Geometry: final body of the model. Coordinates: model frame, mm. Face numbers are marked on the shaded views. A direction names the side the tool comes from. Give positions to 0.01 mm unless a question says otherwise; leave off trailing zeros. Order: outer loops, then holes, each group sorted by start corner. A loop starts at its lowest first (then second) coordinate and runs counter-clockwise, first axis right, second up. Notation, with made-up numbers: (-31, 85) -> (8, 85) arc R33 cw to (8, 119) -> close; hole circle Ø5 at (74.25, 31). An arc over 180 degrees is marked (long way). One line per question, with ' | ' between items.
from build123d import *

# Parameters (mm, degrees)
SKETCH_1_R      = 20
SKETCH_1_R_2    = 14
EXTRUDE_1_DEPTH = 4
SKETCH_2_W      = 40
SKETCH_2_H      = 18
EXTRUDE_2_DEPTH = 2
SKETCH_3_W      = 2
SKETCH_3_H      = 18
EXTRUDE_3_DEPTH = 53
SKETCH_4_W      = 2
SKETCH_4_H      = 18
EXTRUDE_4_DEPTH = 18


with BuildPart() as part:
    # 草图1 → 凸台-拉伸1 (new, symmetric)
    with BuildSketch(Plane.XY):
        Circle(SKETCH_1_R)
        Circle(SKETCH_1_R_2, mode=Mode.SUBTRACT)
    extrude(amount=EXTRUDE_1_DEPTH, both=True)

    # 草图2 → 凸台-拉伸2 (add)
    with BuildSketch(Plane(origin=(0, 0, -4), x_dir=(-1, 0, 0), z_dir=(0, 0, -1))):
        with Locations((37.860571099, 0)):
            Rectangle(SKETCH_2_W, SKETCH_2_H)
    extrude(amount=-EXTRUDE_2_DEPTH)

    # 草图3 → 凸台-拉伸3 (add)
    with BuildSketch(Plane(origin=(0, 0, -4), x_dir=(-1, 0, 0), z_dir=(0, 0, -1))):
        with Locations((56.860571099, 0)):
            Rectangle(SKETCH_3_W, SKETCH_3_H)
    extrude(amount=EXTRUDE_3_DEPTH)

    # 草图4 → 凸台-拉伸4 (add)
    with BuildSketch(Plane.ZY.offset(57.860571099)):
        with Locations((-56, 0)):
            Rectangle(SKETCH_4_W, SKETCH_4_H)
    extrude(amount=EXTRUDE_4_DEPTH)


solid = part.part
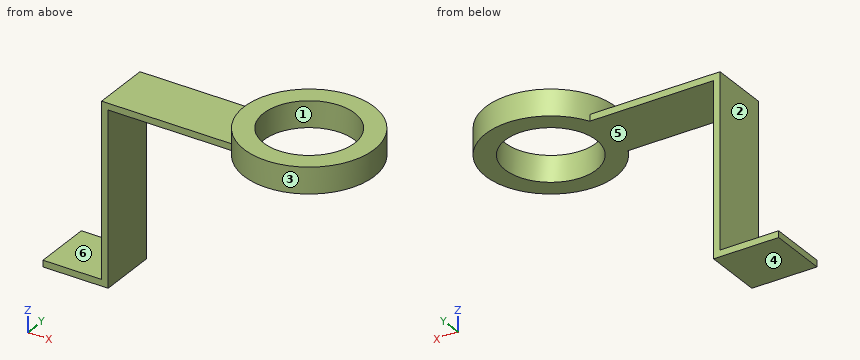
1) Material intervals for probe 1 along Y at (x, z) = (0, -1); probe 2 along Z at (x, y) = (-60, 3); probe 3 along X at (y, z) = (5, -32), sorted ascending. Write a range as from..to.
Check result:
probe 1: y = -20..-14, 14..20 | probe 2: z = -57..-55 | probe 3: x = -57.86..-55.86
2) Section B-B on x = 0. Return loops of the section in (y, z).
Check result:
outline: (-20, -4) -> (-14, -4) -> (-14, 4) -> (-20, 4) -> close; (14, -4) -> (20, -4) -> (20, 4) -> (14, 4) -> close
3) Set-up query: the marked faces 4, 5 and 6. Return all of +Z, -Z, +X, -X, +Y, -Y with unobstructed straight access to the full face (end or side cutting, diameter ignored); none if empty.
Check result:
face 4: -Z, +X, -X, +Y, -Y | face 5: -Z, +X, +Y, -Y | face 6: +Z, -X, +Y, -Y
4) Section D-D on z = -31. Return loops of the section in (x, y), plus the area to 3 significant figures.
Check result:
outline: (-57.86, -9) -> (-55.86, -9) -> (-55.86, 9) -> (-57.86, 9) -> close | area: 36.0 mm^2
5) Section A-A on y = 0. Return loops of the section in (x, z).
Check result:
outline: (-75.86, -57) -> (-55.86, -57) -> (-55.86, -4) -> (-14, -4) -> (-14, 4) -> (-20, 4) -> (-20, -2) -> (-57.86, -2) -> (-57.86, -55) -> (-75.86, -55) -> close; (14, -4) -> (20, -4) -> (20, 4) -> (14, 4) -> close
6) Contact query for flat-ended pins moving along their axis: pin 1 Ø12 at (y, z) = (-7, -13.5) entering from -X; pin 2 Ø16.5 at (x, z) = (-57, -32.5) entering from +Y; pin 3 Ø20 at (x, y) = (-12, -7) entering from -Z. Output: stop coordinate, or through.
Check result:
pin 1: stops at x = -57.86 | pin 2: stops at y = 9 | pin 3: stops at z = -4
7) Section C-C on x = -31. Return loops of the section in (y, z).
Check result:
outline: (-9, -4) -> (9, -4) -> (9, -2) -> (-9, -2) -> close
8) Pull-direction query (X, two-part tool) for the marked faces 1, 2 and 3; classes: +X half, -X half, draft (parallel to the pull), parting line (faces both ways), or undercut.
Check result:
face 1: undercut | face 2: -X half | face 3: parting line
